```python
from build123d import *

# Parameters (mm, degrees)
SKETCH2_W          = 1.97993319
SKETCH2_H          = 2.899664475
CUT_EXTRUDE1_DEPTH = 18
CHAMFER1_SIZE      = 0.5


with BuildPart() as part:
    # Sketch1 → Revolve1 (revolve)
    with BuildSketch(Plane.XY, mode=Mode.PRIVATE) as revolve1_sk:
        Polygon((0, 21.201861416), (-11, 21.201861416), (-11, 16.201861416), (-3, 16.201861416), (-3, -8.798138584), (0, -8.798138584), align=None)
    revolve(revolve1_sk.sketch.rotate(Axis((0, 28.350797586, 0), (0, -1, 0)), 270), axis=Axis((0, 28.350797586, 0), (0, -1, 0)))

    # Sketch2 → Cut-Extrude1 (cut, symmetric)
    with BuildSketch(Plane.XY):
        with Locations((0, 21.201861416)):
            Rectangle(SKETCH2_W, SKETCH2_H)
    extrude(amount=CUT_EXTRUDE1_DEPTH, both=True, mode=Mode.SUBTRACT)

    # Chamfer1
    chamfer1_edges = [part.edges().sort_by_distance(p)[0] for p in [
        (-11, 21.201861416, 0),
        (11, 21.201861416, 0),
    ]]
    chamfer(chamfer1_edges, length=CHAMFER1_SIZE)


solid = part.part
```
Input: part model. Units: mm. Frame: model coordinates. A direction names the side the tool comes from. Round coordinates to 2 decimals unless told otherwise and drop trailing zeros. Loops run counter-clockwise (first coordinate to the right, second up) from the corner with the lowest first, then second, coordinate; pieces in that order, holes last. Notation, with made-up numbers: (6.25, 84) -> (33.25, 84) arc R17 cw to (33.25, 100) -> close; hole circle Ø5 at (13, 45). An arc over 180 degrees is marked (long way). Use one line per item in the form item = value. Start each with the question number.
Item 1: Section query C-C on y = -5. Return the cut outline in (x, z).
Item 2: Contact query for flat-ended pins moving along their axis: pin 1 Ø1.2 at (y, z) = (21, -3) entering from +X; pin 2 Ø1 at (x, y) = (2.5, -5.5) entering from -Z; pin 3 Ø5 at (x, z) = (-6.5, -7) entering from -Y; pin 4 Ø1 at (y, z) = (10.5, 4.5) entering from +X. Output: stop coordinate, or through.
Item 3: Section query A-A on x = 0. Return the cut outline in (y, z).
Item 4: Mould query, pull axis X, two halves, no side actions, for faces 1 (the face through (0.99, 20, 0)), 2 (the face through (-10.64, 21.06, 0.22)), 3 (the face through (0, 19.752, 0)), 4 (the face through (-5, 21.202, 0)). Classes: pulls with the +X half, pulls with the -X half, needs draft (parallel to the pull), parting line crosses it, or undercut.
Item 5: Material intervals for L1, parallel to Y at x = 1.75, z = -10; L2, parallel to Y at x = 0.5, z = -4.5; L3, parallel to Z at x = 9.75, y = 17.5, sorted ascending. Write a range as from..to.
Item 6: Section query B-B on z = 0. Return the cut outline in (x, y), then the cut area to 3 significant figures.
Item 7: Set-up query: faces 5 (the face through (0, -8.798, 0)), 6 (the face through (-0.99, 20, 0)), 7 (the face through (2.3, 16.202, 2.3)). Return all of +Z, -Z, +X, -X, +Y, -Y with unobstructed straight access to the full face (end or side cutting, diameter ignored); none if empty.
Ans:
q1.outline = circle Ø6 at (0, 0)
q2.pin_1 = 10.72
q2.pin_2 = -2.24
q2.pin_3 = 16.2
q2.pin_4 = through
q3.outline = (-8.8, -3) -> (16.2, -3) -> (16.2, -11) -> (19.75, -11) -> (19.75, 11) -> (16.2, 11) -> (16.2, 3) -> (-8.8, 3) -> close
q4.face_1 = undercut
q4.face_2 = pulls with the -X half
q4.face_3 = undercut
q4.face_4 = needs draft
q5.L1 = 16.2..21.2
q5.L2 = 16.2..19.75
q5.L3 = -5.09..5.09
q6.outline = (-11, 16.2) -> (-3, 16.2) -> (-3, -8.8) -> (3, -8.8) -> (3, 16.2) -> (11, 16.2) -> (11, 20.7) -> (10.5, 21.2) -> (0.99, 21.2) -> (0.99, 19.75) -> (-0.99, 19.75) -> (-0.99, 21.2) -> (-10.5, 21.2) -> (-11, 20.7) -> close
q6.area = 257 mm^2
q7.face_5 = +Z, -Z, +X, -X, -Y
q7.face_6 = +Z, -Z, +Y
q7.face_7 = -Y
